Part model, mm, in its own coordinate system. Face numbers are marked on the shaded views. A direction names the side the tool comes from. Round coordinates to 2 decimals unless told otherwise and drop trailing zeros. Order: outer loops, then holes, each group sorted by start corner. A loop starts at its lowest first (then second) coordinate and runs counter-clockwise, first axis right, second up. Notation, with made-up numbers: (-39.75, -31) -> (-23.75, -31) arc R25 cw to (-23.75, 2) -> close; hole circle Ø5 at (-37, 10.5). An arc over 180 degrees is marked (long way). Return JSON: item names as keys, results as strings. Group by question number.
from build123d import *

# Parameters (mm, degrees)
SKETCH_1_R                  = 10
EXTRUDE_1_DEPTH             = 7.5
HOLE_WIZARD_2_D             = 9
HOLE_WIZARD_2_CBORE_D       = 15
HOLE_WIZARD_2_CBORE_DEPTH   = 9
CHAMFER_1_SIZE              = 1
PATTERN_CIRCULAR_1_COUNT    = 8
HOLE_WIZARD_2_2_D           = 3.4
HOLE_WIZARD_2_2_CBORE_D     = 6
HOLE_WIZARD_2_2_CBORE_DEPTH = 3.4
HOLE_WIZARD_8_0_8_1_D       = 8
HOLE_WIZARD_8_0_8_1_DEPTH   = 8
HOLE_WIZARD_8_0_8_1_TIP     = 2.403442476
HOLE_WIZARD_M4_1_D          = 3.3
SKETCH_10_W                 = 135
SKETCH_10_H                 = 15
CUT_EXTRUDE_1_DEPTH         = 3
HOLE_WIZARD_3_D             = 6.6
HOLE_WIZARD_3_CBORE_D       = 11
HOLE_WIZARD_3_CBORE_DEPTH   = 6.8
CHAMFER_2_SIZE              = 3


with BuildPart() as part:
    # 草图1 → 凸台-拉伸1 (new, symmetric)
    with BuildSketch(Plane.XY):
        with BuildLine():
            Line((-55.784271247, -9.215728753), (-34.215728753, -30.784271247))
            ThreePointArc((-34.215728753, -30.784271247), (-21.2387948, -39.4551813), (-5.931457505, -42.5))
            Line((-5.931457505, -42.5), (5.931457505, -42.5))
            ThreePointArc((5.931457505, -42.5), (21.2387948, -39.4551813), (34.215728753, -30.784271247))
            Line((34.215728753, -30.784271247), (55.784271247, -9.215728753))
            ThreePointArc((55.784271247, -9.215728753), (64.4551813, 3.7612052), (67.5, 19.068542495))
            Line((67.5, 19.068542495), (67.5, 42.5))
            Line((67.5, 42.5), (-67.5, 42.5))
            Line((-67.5, 42.5), (-67.5, 19.068542495))
            ThreePointArc((-67.5, 19.068542495), (-64.4551813, 3.7612052), (-55.784271247, -9.215728753))
        make_face()
        Circle(SKETCH_1_R, mode=Mode.SUBTRACT)
    extrude(amount=EXTRUDE_1_DEPTH, both=True)

    # Hole Wizard 2 (through all)
    with Locations(Plane.XY.offset(7.5)):
        with Locations((-8.03635208, 19.401470183)):
            hole_wizard_2 = CounterBoreHole(HOLE_WIZARD_2_D / 2, HOLE_WIZARD_2_CBORE_D / 2, HOLE_WIZARD_2_CBORE_DEPTH)

    # 倒角1
    chamfer_1_edges = [part.edges().sort_by_distance(p)[0] for p in [
        (-10, 0, -7.5),
        (-10, 0, 7.5),
    ]]
    chamfer(chamfer_1_edges, length=CHAMFER_1_SIZE)

    # 阵列(圆周)1: Hole Wizard 2 ×8 about axis
    pattern_circular_1_axis = Axis((0, 0, 0), (0, 0, 1))
    for i in range(1, PATTERN_CIRCULAR_1_COUNT):
        add(hole_wizard_2.rotate(pattern_circular_1_axis, i * 360 / PATTERN_CIRCULAR_1_COUNT), mode=Mode.SUBTRACT)

    # Hole Wizard 2 2 (through all)
    with Locations(Plane.XY.offset(7.5)):
        with Locations((-54, 0), (54, 0)):
            CounterBoreHole(HOLE_WIZARD_2_2_D / 2, HOLE_WIZARD_2_2_CBORE_D / 2, HOLE_WIZARD_2_2_CBORE_DEPTH)

    # Ø8.0 (8) 直径孔1
    with Locations(Plane(origin=(0, 0, -7.5), x_dir=(-1, 0, 0), z_dir=(0, 0, -1))):
        with Locations((-54, 0), (54, 0)):
            Hole(HOLE_WIZARD_8_0_8_1_D / 2, depth=HOLE_WIZARD_8_0_8_1_DEPTH)
            with Locations((0, 0, -(HOLE_WIZARD_8_0_8_1_DEPTH + HOLE_WIZARD_8_0_8_1_TIP / 2))):  # 118° drill point
                Cone(0, HOLE_WIZARD_8_0_8_1_D / 2, HOLE_WIZARD_8_0_8_1_TIP, mode=Mode.SUBTRACT)

    # M4 螺纹孔1 (through all)
    with Locations(Plane(origin=(0, 0, -7.5), x_dir=(-1, 0, 0), z_dir=(0, 0, -1))):
        with Locations((-14, 0), (14, 0)):
            Hole(HOLE_WIZARD_M4_1_D / 2)

    # 草图10 → 切除-拉伸1 (cut)
    with BuildSketch(Plane.XY.offset(7.5)):
        with Locations((0, 35)):
            Rectangle(SKETCH_10_W, SKETCH_10_H)
    extrude(amount=-CUT_EXTRUDE_1_DEPTH, mode=Mode.SUBTRACT)

    # 打孔尺寸(%根据)内六角圆柱头螺钉的类型3 (through all)
    with Locations(Plane(origin=(0, 0, -7.5), x_dir=(-1, 0, 0), z_dir=(0, 0, -1))):
        with Locations((-20, 35), (-60, 35), (60, 35), (20, 35)):
            CounterBoreHole(HOLE_WIZARD_3_D / 2, HOLE_WIZARD_3_CBORE_D / 2, HOLE_WIZARD_3_CBORE_DEPTH)

    # 倒角2
    chamfer_2_edges = [part.edges().sort_by_distance(p)[0] for p in [
        (-67.5, 42.5, -1.5),
        (67.5, 42.5, -1.5),
    ]]
    chamfer(chamfer_2_edges, length=CHAMFER_2_SIZE)


solid = part.part
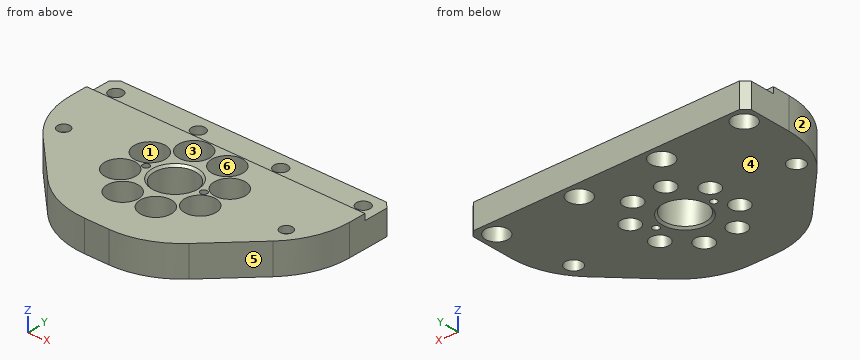
(1) Saw through at C-C, the plane y = 8. State how many separate pieces and enclosed holes the cut face has, and give its area (3 significant figures).
(2) Saw through at B-B, the plane x = 38. List the corners of the cut face in (y, z), and give its area (4 significant figures).
(3) Probe L1, parallel to Y at x = 54, z = 5.4; L2, parallel to X at y = -7, z = 1.75; L3, parallel to X at y = -8.5, z = 2.5. List the from-to ranges inside material, lowest first. Write a range as [from, to].
(4) Mould opens along Y. For the marked faces 1, 2, 3 and 4 say: pulls with the +Y half, pulls with the -Y half, needs draft (parallel to the pull), parting line crosses it, or undercut.
(5) Pin check, flat tips, straight feed: P1, Ø6.5, axis at x = -54, y = 0, coming from the +Z side; P2, Ø1.5, axis at y = -29, z = -3.5, coming from the -X side; P3, Ø12, axis at x = -8.04, y = -19.4, coming from the +Z side; P4, Ø10, axis at x = -60, y = 35, coming from the -Z side. Stop position of each tip, or through.
(6) Tool access for the marked faces 5 and 6: list every direction of +Z, -Z, +X, -X, +Y, -Y with a clear straight run to the whole face (end or side of a thin tool).
(7) Saw through at A-A, the plane x = -60. List the corners of the cut face in (y, z).
Results are:
{
 "1": {"separate pieces": "4", "enclosed holes": "0", "area": "1,420 mm^2"},
 "2": {"outline": "(-27, -7.5) -> (42.5, -7.5) -> (42.5, 4.5) -> (27.5, 4.5) -> (27.5, 7.5) -> (-27, 7.5) -> close", "area": "997.5 mm^2"},
 "3": {"L1": "y = [-11, -3], [3, 27.5]", "L2": "x = [-57.84, -26.83], [-11.97, -7.14], [7.14, 11.97], [26.83, 57.84]", "L3": "x = [-56.48, -26.89], [-11.92, -5.27], [5.27, 11.92], [26.89, 56.48]"},
 "4": {"face 1": "undercut", "face 2": "pulls with the -Y half", "face 3": "undercut", "face 4": "needs draft"},
 "5": {"P1": "stops at z = 7.5", "P2": "stops at x = -36.75", "P3": "stops at z = -1.5", "P4": "stops at z = -0.7"},
 "6": {"face 5": "+Z, -Z, +X, -Y", "face 6": "+Z"},
 "7": {"outline": "(-4.25, -7.5) -> (29.5, -7.5) -> (29.5, -0.7) -> (31.7, -0.7) -> (31.7, 4.5) -> (27.5, 4.5) -> (27.5, 7.5) -> (-4.25, 7.5) -> close; (38.3, -0.7) -> (40.5, -0.7) -> (40.5, -7.5) -> (42.5, -7.5) -> (42.5, 4.5) -> (38.3, 4.5) -> close"}
}
